Study the drawing (mm; zero at the part's minimum x, y, z) and answer. Coordinates: 2 decimals unless noted, no trailing zeros. Loops run counter-clockwise (first coordinate to the right, second up) from the corner with the lowest first, then second, coordinate; pieces in that order, holes last. Notation, with made-up numbers: (28.25, 62) - (71.25, 62) arc R21 ccw to (71.25, 101) - close; hole circle Ø10 at (57, 40). An arc over 180 degrees is marked (long way). Use one line per item in the form item = value.
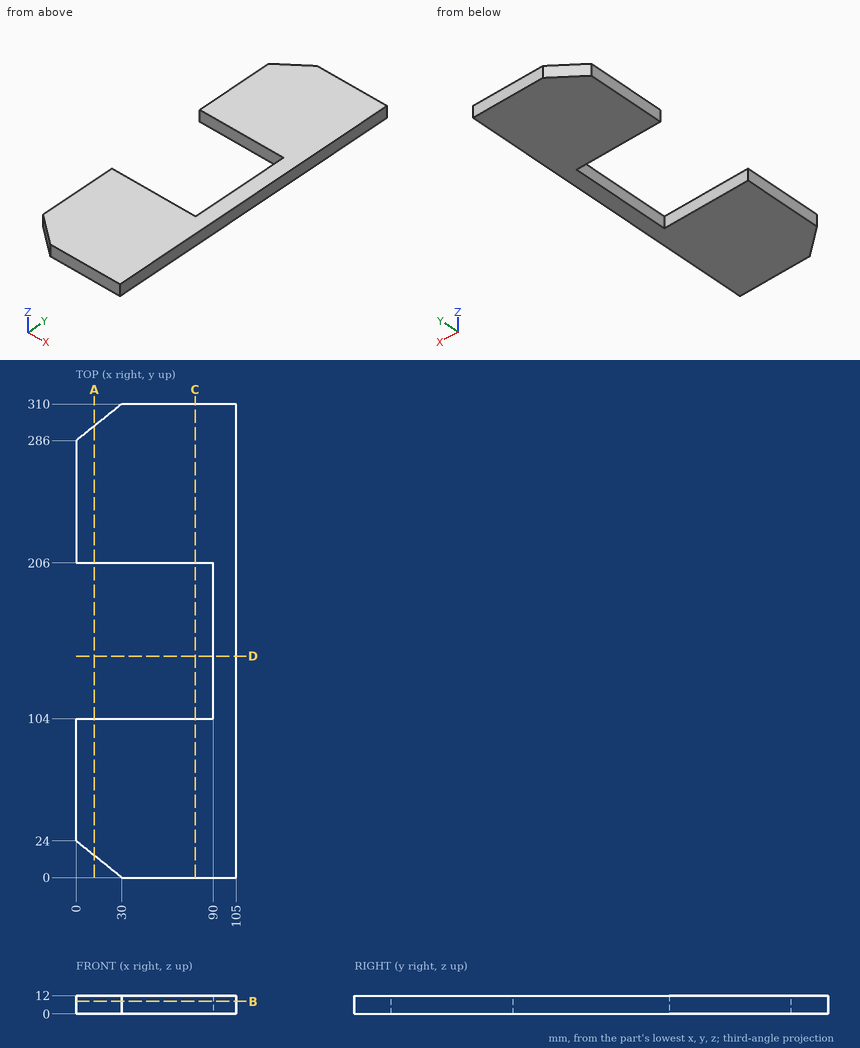
Item 1: The part is cut by section B-B on z = 8.25. Give the vertices of the cut face in (x, y), plus the area to 4 significant figures.
Results below:
outline = (0, 24) - (30, 0) - (105, 0) - (105, 310) - (30, 310) - (0, 286) - (0, 206) - (90, 206) - (90, 104) - (0, 104) - close
area = 22,650 mm²
Item 2: This flat-tipped pin is pushed along its axis until it touches: P1, Ø3.5, axis at y = 180, z = 3.5, coming from the -X side. Where does it stop, or does it pass through?
Results below:
P1 = 90
Item 3: The part is cut by section C-C on x = 78. Give the vertices of the cut face in (y, z).
Results below:
outline = (0, 0) - (104, 0) - (104, 12) - (0, 12) - close; (206, 0) - (310, 0) - (310, 12) - (206, 12) - close
Item 4: The part is cut by section A-A on x = 12. Give the vertices of the cut face in (y, z).
Results below:
outline = (14.4, 0) - (104, 0) - (104, 12) - (14.4, 12) - close; (206, 0) - (295.6, 0) - (295.6, 12) - (206, 12) - close
Item 5: Find the intervals of material crossed by L1, parallel to Y at x = 83.5, z = 7.75; L2, parallel to X at y = 147.5, z = 11.75; L3, parallel to Y at x = 19, z = 10.75, in increasing order.
Results below:
L1 = 0 to 104, 206 to 310
L2 = 90 to 105
L3 = 8.8 to 104, 206 to 301.2
Item 6: The part is cut by section D-D on y = 145. Give the vertices of the cut face in (x, z), plus the area to 3 significant figures.
Results below:
outline = (90, 0) - (105, 0) - (105, 12) - (90, 12) - close
area = 180 mm²
